from build123d import *

# Parameters (mm, degrees)
SKETCH1_R           = 6.499999992
BOSS_EXTRUDE1_DEPTH = 6
SKETCH2_R           = 3
CUT_EXTRUDE1_DEPTH  = 12


with BuildPart() as part:
    # Sketch1 → Boss-Extrude1 (new, symmetric)
    with BuildSketch(Plane.XY):
        with BuildLine():
            Line((249.080198754, 296.842221709), (267.033227589, 318.237808321))
            ThreePointArc((267.033227589, 318.237808321), (295.209868645, 320.702944991), (297.675005315, 292.526303935))
            Line((297.675005315, 292.526303935), (278.391377025, 269.544970642))
            ThreePointArc((278.391377025, 269.544970642), (264.088717655, 283.572564272), (249.080198754, 296.842221709))
        make_face()
        with Locations((282.354116452, 305.382056128)):
            Circle(SKETCH1_R, mode=Mode.SUBTRACT)
    extrude(amount=BOSS_EXTRUDE1_DEPTH, both=True)

    # Sketch2 → Cut-Extrude1 (cut)
    with BuildSketch(Plane(origin=(0, 0, -6), x_dir=(-1, 0, 0), z_dir=(0, 0, -1))):
        with Locations(Location((-291.674536792, 316.489700554, 0), (0, 0, 90))):
            Circle(SKETCH2_R)
        with Locations(Location((-271.246472026, 314.702476468, 0), (0, 0, 90))):
            Circle(SKETCH2_R)
        with Locations(Location((-273.033696112, 294.274411702, 0), (0, 0, 90))):
            Circle(SKETCH2_R)
    extrude(amount=-CUT_EXTRUDE1_DEPTH, mode=Mode.SUBTRACT)


solid = part.part
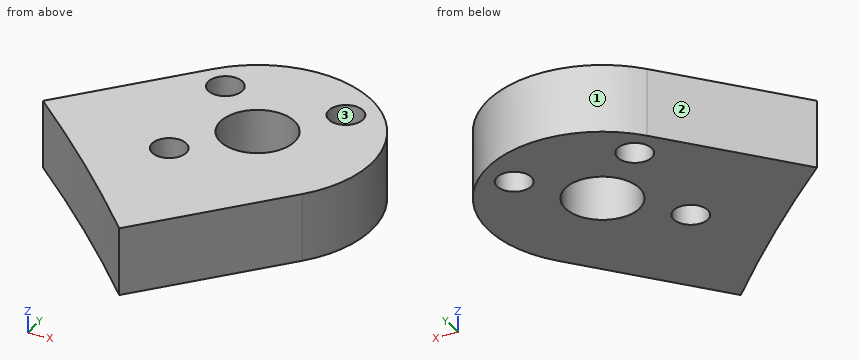
Could you check a few things on this model? Use its own coordinates, in mm. Face numbers are marked on the shaded views. Give positions to 0.01 mm unless a question says otherwise; leave off trailing zeros. Order: outer loops, then holes, each group sorted by start corner. A loop starts at its lowest first (then second) coordinate and runs counter-clockwise, first axis right, second up. Notation, with made-up numbers: (14.5, 84.25) -> (39.5, 84.25) arc R30 cw to (39.5, 119.25) -> close; hole circle Ø3 at (17.5, 47). An arc over 180 degrees is marked (long way). Answer in a Markdown table with one row per item. Add a question column.
Item 1: Imagine slicing it at B-B (x = 281). List the corners of the cut face in (y, z) for me, and give its area (3 significant figures).
Item 2: Imagine slicing it at C-C (z = -2.5). List the corners of the cut face in (x, y) for me (3 decimals).
Item 3: Please list where these lines run through material, in increasing order: probe 1 along Y at (x, z) = (272.5, -4.75); probe 2 along Y at (x, z) = (274, 3); probe 3 along X at (y, z) = (315, 2.25).
Item 4: I'm going to push flat-ended pins straight in: P1, Ø5.5, axis at x = 271.25, y = 314.7, coming from the -Z side; P2, Ø4, axis at y = 276, z = -2, coming from the -X side; P3, Ø1, axis at y = 304.5, z = -4, coming from the +X side; P4, Ø2, axis at y = 294.5, z = 3, coming from the +X side. Where does each tip first touch, or does it pass through?
Item 5: Imagine slicing it at A-A (y = 309.5). List the corners of the cut face in (x, z) for me, and give its area (3 significant figures).
Item 6: We'd pull the mould along X, two halves only. Please class the marked faces 1, 2 and 3: pulls with the +X half, pulls with the -X half, needs draft (parallel to the pull), parting line crosses it, or undercut.
Item 7: Imagine slicing it at D-D (x = 272). List the corners of the cut face in (y, z) for me, and give its area (3 significant figures).
Result:
| question | item | result |
|---|---|---|
| 1 | outline | (272.65, -6) -> (299.02, -6) -> (299.02, 6) -> (272.65, 6) -> close; (311.74, -6) -> (325.34, -6) -> (325.34, 6) -> (311.74, 6) -> close |
| 1 | area | 480 mm2 |
| 2 | outline | (249.08, 296.842) arc R387.5 cw to (278.391, 269.545) -> (297.675, 292.526) arc R20 ccw to (267.033, 318.238) -> close; hole circle Ø6 at (271.246, 314.702); hole circle Ø6 at (273.034, 294.274); hole circle Ø13 at (282.354, 305.382); hole circle Ø6 at (291.675, 316.49) |
| 3 | probe 1 | 275.5 to 291.32, 297.23 to 311.98, 317.43 to 322.79 |
| 3 | probe 2 | 274.01 to 291.43, 297.11 to 313.51, 315.89 to 323.55 |
| 3 | probe 3 | 264.32 to 268.26, 274.23 to 289.07, 294.28 to 299.89 |
| 4 | P1 | through |
| 4 | P2 | x = 269.95 |
| 4 | P3 | x = 302.35 |
| 4 | P4 | x = 299.74 |
| 5 | outline | (259.7, -6) -> (277.32, -6) -> (277.32, 6) -> (259.7, 6) -> close; (287.38, -6) -> (301.93, -6) -> (301.93, 6) -> (287.38, 6) -> close |
| 5 | area | 386 mm2 |
| 6 | face 1 | parting line crosses it |
| 6 | face 2 | pulls with the -X half |
| 6 | face 3 | undercut |
| 7 | outline | (275.99, -6) -> (291.46, -6) -> (291.46, 6) -> (275.99, 6) -> close; (297.09, -6) -> (311.8, -6) -> (311.8, 6) -> (297.09, 6) -> close; (317.61, -6) -> (322.49, -6) -> (322.49, 6) -> (317.61, 6) -> close |
| 7 | area | 421 mm2 |
